from build123d import *

# Parameters (mm, degrees)
SKETCH1_W                                           = 16.5
SKETCH1_H                                           = 15
BOSS_EXTRUDE1_DEPTH                                 = 18
FILLET1_R                                           = 1
CBORE_FOR_M4_HEX_SOCKET_HEAD_CAP_SCREW1_D           = 4.5
CBORE_FOR_M4_HEX_SOCKET_HEAD_CAP_SCREW1_CBORE_D     = 7.5
CBORE_FOR_M4_HEX_SOCKET_HEAD_CAP_SCREW1_CBORE_DEPTH = 8
SKETCH7_R                                           = 16
CUT_EXTRUDE2_DEPTH                                  = 22.17339132
SKETCH8_W                                           = 6.5
SKETCH8_H                                           = 12
CUT_EXTRUDE3_DEPTH                                  = 25.840742743
SKETCH9_W                                           = 10
SKETCH9_H                                           = 12
CUT_EXTRUDE4_DEPTH                                  = 2.5
FILLET2_R                                           = 1


with BuildPart() as part:
    # Sketch1 → Boss-Extrude1 (new body)
    with BuildSketch(Plane.XY):
        Rectangle(SKETCH1_W, SKETCH1_H)
    extrude(amount=BOSS_EXTRUDE1_DEPTH)

    # Fillet1
    fillet1_edges = [part.edges().sort_by_distance(p)[0] for p in [
        (-8.25, -7.5, 9),
        (-8.25, 7.5, 9),
    ]]
    fillet(fillet1_edges, radius=FILLET1_R)

    # CBORE for M4 Hex Socket Head Cap Screw1 (through all)
    with Locations(Plane.XY.offset(18)):
        with Locations((-2.75, 0)):
            CounterBoreHole(CBORE_FOR_M4_HEX_SOCKET_HEAD_CAP_SCREW1_D / 2, CBORE_FOR_M4_HEX_SOCKET_HEAD_CAP_SCREW1_CBORE_D / 2, CBORE_FOR_M4_HEX_SOCKET_HEAD_CAP_SCREW1_CBORE_DEPTH)

    # Sketch7 → Cut-Extrude2 (cut, through all)
    with BuildSketch(Plane.XY.offset(18)):
        with Locations((22.25, 0)):
            Circle(SKETCH7_R)
    extrude(amount=-CUT_EXTRUDE2_DEPTH, mode=Mode.SUBTRACT)

    # Sketch8 → Cut-Extrude3 (cut, through all)
    with BuildSketch(Plane(origin=(0, 7.5, 0), x_dir=(1, 0, 0), z_dir=(0, 1, 0))):
        with Locations((5, -6)):
            Rectangle(SKETCH8_W, SKETCH8_H)
    extrude(amount=-CUT_EXTRUDE3_DEPTH, mode=Mode.SUBTRACT)

    # Sketch9 → Cut-Extrude4 (cut)
    with BuildSketch(Plane(origin=(0, -7.5, 0), x_dir=(-1, 0, 0), z_dir=(0, -1, 0))):
        with Locations((3.25, -6)):
            Rectangle(SKETCH9_W, SKETCH9_H)
    cut_extrude4 = extrude(amount=-CUT_EXTRUDE4_DEPTH, mode=Mode.SUBTRACT)

    # Mirror1: Cut-Extrude4 across plane
    add(cut_extrude4.mirror(Plane.ZX), mode=Mode.SUBTRACT)

    # Fillet2
    fillet2_edges = [part.edges().sort_by_distance(p)[0] for p in [
        (-8.25, 5, 6),
        (-8.25, -5, 6),
    ]]
    fillet(fillet2_edges, radius=FILLET2_R)


solid = part.part
Check sheet for the modelled part. Datum: model origin and axes. Units: mm. A direction names the side the tool comes from. Coordinates: 2 decimals unless noted, no trailing zeros. Write each loop counter-clockwise with the first axis right and the second up, starting at its lowest first coordinate (ties: lowest second). Pieces come first, ordered by that corner, then holes.
Item 1: Depth check by flat-ended pin: pin 1 Ø4.5 at (x, z) = (-2.5, 7) entering from -Y; pin 2 Ø2 at (x, y) = (-3, 1.5) entering from +Z. Enter the tip coordinate at first touch or a pass-through.
Numbers:
pin 1: stops at y = -5
pin 2: stops at z = 10
Item 2: Scan lines: probe 1 along Y at (x, z) = (-2.75, 12.75); probe 2 along Y at (x, z) = (-2.75, 5.75); probe 3 along Z at (x, y) = (0.5, -5.25). Record each from-to range of solid material in increasing order.
Numbers:
probe 1: y = -7.5 to -3.75, 3.75 to 7.5
probe 2: y = -5 to -2.25, 2.25 to 5
probe 3: z = 12 to 18
Item 3: Mould release check, pull along X, two halves, no side actions. Record for faces 5 (the face through (2, 0, 18)), 6 (the face through (-1, -2, 10)), 7 (the face through (-7.965, -7.199, 15.042)): released by +X, released by -X, zero draft, split by the parting line, or undercut.
Numbers:
face 5: zero draft
face 6: undercut
face 7: released by -X
Item 4: Cross-section at A-A on y = 0. Record the boundary of the cut face in (x, z).
Numbers:
outline: (-8.25, 0) - (-5, 0) - (-5, 10) - (-6.5, 10) - (-6.5, 18) - (-8.25, 18) - close; (-0.5, 0) - (1.75, 0) - (1.75, 12) - (6.25, 12) - (6.25, 18) - (1, 18) - (1, 10) - (-0.5, 10) - close
Item 5: Cross-section at B-B on x = -2.75. Record the boundary of the cut face in (y, z), then the cut area to 3 significant figures.
Numbers:
outline: (-7.5, 12) - (-5, 12) - (-5, 0) - (-2.25, 0) - (-2.25, 10) - (-3.75, 10) - (-3.75, 18) - (-7.5, 18) - close; (2.25, 0) - (5, 0) - (5, 12) - (7.5, 12) - (7.5, 18) - (3.75, 18) - (3.75, 10) - (2.25, 10) - close
area: 105 mm2
Item 6: Cross-section at C-C on z = 2. Record the boundary of the cut face in (x, y).
Numbers:
outline: (-8.25, -4) arc R1 ccw to (-7.25, -5) - (1.75, -5) - (1.75, 5) - (-7.25, 5) arc R1 ccw to (-8.25, 4) - close; hole circle Ø4.5 at (-2.75, 0)
Item 7: Cross-section at D-D on y = 3.5. Record the boundary of the cut face in (x, z), then the cut area to 3 significant figures.
Numbers:
outline: (-8.25, 0) - (1.75, 0) - (1.75, 12) - (6.64, 12) - (6.64, 18) - (-1.4, 18) - (-1.4, 10) - (-4.1, 10) - (-4.1, 18) - (-8.25, 18) - close
area: 188 mm2
Item 8: Access from +Z, -Z, +X, -X, +Y, -Y to the whole of each face (thin tool, end or side, straight path). Record for faces 1 (the face through (-7.965, -4.699, 5.916)), 2 (the face through (-6.496, 0.165, 14.056)), 3 (the face through (-7.965, 4.699, 5.916)), 4 (the face through (-3, 5, 6)).
Numbers:
face 1: -Z, -X, -Y
face 2: +Z
face 3: -Z, -X, +Y
face 4: -Z, +X, -X, +Y
